Read the model definition and answer for the solid it produces. Units are mm, in the model's axes. Coordinates: 2 decimals unless noted, no trailing zeros. Loops run counter-clockwise (first coordinate to the right, second up) from the corner with the lowest first, then second, coordinate; pieces in that order, holes last. Notation, with made-up numbers: (-31.75, -15) -> (-10.75, -15) arc R26 ccw to (-10.75, 1) -> close; hole circle Ø9 at (78, 33). An arc over 180 degrees is marked (long way). Answer as a JSON object with one key per item and string values. Group by question number.
Q1. Straight lines are drawn through the part: line 1 along Y through (x, z) = (49, 1.3); line 2 along Y through (x, z) = (47.5, 1.2); line 3 along Y through (x, z) = (126, 0.6). For each, find the intervals that lie inside material, in ascending order. Write a range as [from, to].
Q2. Each of these flat-tipped pins is pushed along its axis until it touches: P1, Ø17.5, axis at x = 48.41, y = -16.55, coming from the +Z side; P2, Ø1, axis at x = 249, z = 0.5, coming from the -Y side. Where does it stop, or does it pass through?
Q3. The part is cut by section C-C on y = 49. Write down the section's boundary in (x, z).
Q4. The part is cut by section B-B on x = 106. Write down the section's boundary in (y, z).
Q5. The part is cut by section A-A on z = 1.35. Write down the section's boundary in (x, y).
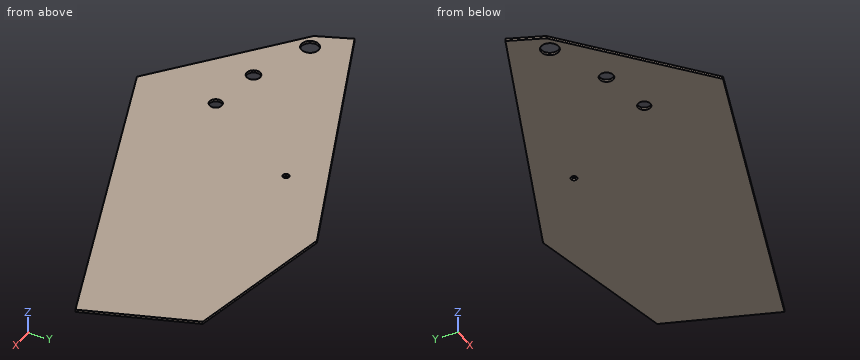
from build123d import *

# Parameters (mm, degrees)
SKETCH_1_R          = 3
EXTRUDE_1_DEPTH     = 2
EXTRUDE_2_DEPTH     = 2
SKETCH_4_OUTSIDE_W  = 464.3
SKETCH_4_OUTSIDE_H  = 281.017
CUT_EXTRUDE_1_DEPTH = 10
EXTRUDE_3_DEPTH     = 2
SKETCH_6_R          = 7
CUT_EXTRUDE_2_DEPTH = 16
EXTRUDE_4_DEPTH     = 2
CUT_EXTRUDE_3_DEPTH = 10
CUT_EXTRUDE_4_DEPTH = 10
SKETCH_10_R         = 2.5
CUT_EXTRUDE_5_DEPTH = 369.29137958
SKETCH_11_R         = 5.5
CUT_EXTRUDE_6_DEPTH = 369.29137958
SKETCH_13_R         = 5
CUT_EXTRUDE_7_DEPTH = 369.29137958


with BuildPart() as part:
    # 草图1 → 凸台-拉伸1 (new body)
    with BuildSketch(Plane.XY):
        with BuildLine():
            Line((362.493953978, 12.044043029), (89.890291348, -87.17557592))
            Line((89.890291348, -87.17557592), (-5.785088487, -6.894399988))
            ThreePointArc((-5.785088487, -6.894399988), (-6.894399988, 5.785088487), (5.785088487, 6.894399988))
            Line((5.785088487, 6.894399988), (93.499500944, -66.706731154))
            Line((93.499500944, -66.706731154), (356.337591398, 28.958510203))
            ThreePointArc((356.337591398, 28.958510203), (367.873006275, 23.579457906), (362.493953978, 12.044043029))
        make_face()
        with Locations((359.415772688, 20.501276616)):
            Circle(SKETCH_1_R, mode=Mode.SUBTRACT)
        Circle(SKETCH_1_R, mode=Mode.SUBTRACT)
    extrude(amount=EXTRUDE_1_DEPTH)

    # 草图3 → 凸台-拉伸2 (add)
    with BuildSketch(Plane.XY.offset(2)):
        Polygon((24.555501063, -8.855846282), (93.499500944, -66.706731154), (337.819582349, 22.218506111), (302.512305891, 106.957456662), align=None)
    extrude(amount=-EXTRUDE_2_DEPTH)

    # 草图4 outside → 切除-拉伸1 (cut)
    with BuildSketch(Plane(origin=(0, 0, 0), x_dir=(-1, 0, 0), z_dir=(0, 0, -1))):
        with Locations((-179.708, 9.8905)):
            Rectangle(SKETCH_4_OUTSIDE_W, SKETCH_4_OUTSIDE_H)
        Polygon((-337.819582349, 22.218506111), (-344.749797365, 5.585698189), (-89.890291348, -87.17557592), (-5.843844232, -16.652233143), (-24.555501063, -8.855846282), (-302.512305891, 106.957456662), align=None, mode=Mode.SUBTRACT)
    extrude(amount=-CUT_EXTRUDE_1_DEPTH, mode=Mode.SUBTRACT)

    # 草图5 → 凸台-拉伸3 (add)
    with BuildSketch(Plane(origin=(0, 0, 0), x_dir=(-1, 0, 0), z_dir=(0, 0, -1))):
        Polygon((-302.512305891, 106.957456662), (-283.449488043, 152.709022376), (-92.70915772, 73.235279423), (36.914573348, 19.226339278), (-5.843844232, -16.652233143), align=None)
    extrude(amount=-EXTRUDE_3_DEPTH)

    # 草图6 → 切除-拉伸2 (cut)
    with BuildSketch(Plane(origin=(0, 0, 0), x_dir=(-1, 0, 0), z_dir=(0, 0, -1))):
        with Locations((-0.401023288, 2.274316085)):
            Circle(SKETCH_6_R)
    extrude(amount=-CUT_EXTRUDE_2_DEPTH, mode=Mode.SUBTRACT)

    # 草图7 → 凸台-拉伸4 (add)
    with BuildSketch(Plane(origin=(0, 0, 0), x_dir=(-1, 0, 0), z_dir=(0, 0, -1))):
        Polygon((-344.749797365, 5.585698189), (-349.390825639, 7.274894338), (-348.706785352, 9.154279579), (-294.744261489, 157.415095392), (-283.449488043, 152.709022376), align=None)
    extrude(amount=-EXTRUDE_4_DEPTH)

    # 草图8 → 切除-拉伸3 (cut)
    with BuildSketch(Plane.XY.offset(2)):
        Polygon((318.426035297, 92.349956602), (196.426191084, 116.449951619), (294.744261489, 157.415095392), align=None)
    extrude(amount=-CUT_EXTRUDE_3_DEPTH, mode=Mode.SUBTRACT)

    # 草图9 → 切除-拉伸4 (cut)
    with BuildSketch(Plane(origin=(0, 0, 0), x_dir=(-1, 0, 0), z_dir=(0, 0, -1))):
        Polygon((23.068383558, 24.995483781), (11.929294577, -1.738798924), (36.914573348, 19.226339278), align=None)
    extrude(amount=-CUT_EXTRUDE_4_DEPTH, mode=Mode.SUBTRACT)

    # 草图10 → 切除-拉伸5 (cut, through all)
    with BuildSketch(Plane.XY.offset(2)):
        with Locations((140.777993137, 60.76369374)):
            Circle(SKETCH_10_R)
    extrude(amount=-CUT_EXTRUDE_5_DEPTH, mode=Mode.SUBTRACT)

    # 草图11 → 切除-拉伸6 (cut, through all)
    with BuildSketch(Plane(origin=(0, 0, 0), x_dir=(-1, 0, 0), z_dir=(0, 0, -1))):
        with Locations((-48.407364973, -16.547379186)):
            Circle(SKETCH_11_R)
    extrude(amount=-CUT_EXTRUDE_6_DEPTH, mode=Mode.SUBTRACT)

    # 草图13 → 切除-拉伸7 (cut, through all)
    with BuildSketch(Plane(origin=(0, 0, 0), x_dir=(-1, 0, 0), z_dir=(0, 0, -1))):
        with Locations((-90.449951862, -23.568027643)):
            Circle(SKETCH_13_R)
    extrude(amount=-CUT_EXTRUDE_7_DEPTH, mode=Mode.SUBTRACT)


solid = part.part
Final values:
{
 "1": {"line 1": "y = [-52.86, -22.02], [-11.08, 55.02]", "line 2": "y = [-51.61, -21.97], [-11.12, 54.4]", "line 3": "y = [-74.03, 87.11]"},
 "2": {"P1": "stops at z = 2", "P2": "stops at y = -29.45"},
 "3": {"outline": "(34.54, 0) -> (334.2, 0) -> (334.2, 2) -> (34.54, 2) -> close"},
 "4": {"outline": "(-81.31, 0) -> (78.77, 0) -> (78.77, 2) -> (-81.31, 2) -> close"},
 "5": {"outline": "(-23.07, 25) -> (-11.93, -1.74) -> (89.89, -87.18) -> (349.39, 7.27) -> (318.43, 92.35) -> (196.43, 116.45) -> close; hole circle Ø14 at (0.4, 2.27); hole circle Ø11 at (48.41, -16.55); hole circle Ø10 at (90.45, -23.57); hole circle Ø5 at (140.78, 60.76)"}
}
